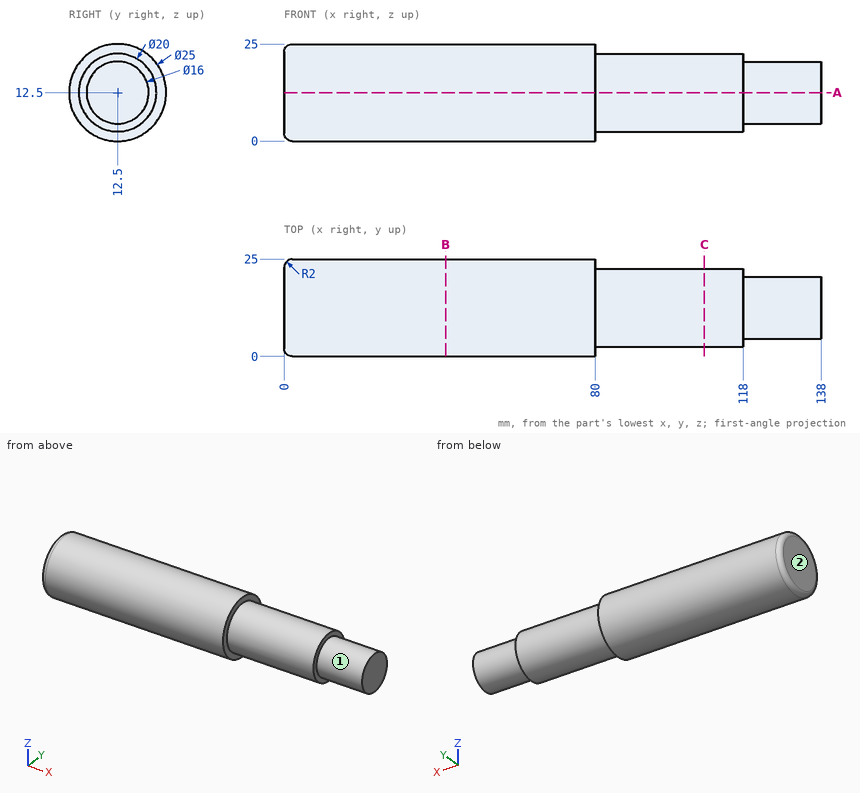
Job drawing, mm, ordinate dimensions from the low corner. One solid piece. A direction names the side the tool comes from. Round coordinates to 2 decimals unless told otherwise and drop trailing zeros. Order: outer loops, then holes, each group sorted by start corner. A loop starts at its lowest first (then second) coordinate and runs counter-clockwise, first axis right, second up. Notation, with made-up numbers: M 53.25,73.5 L 70.25,73.5 A11 ccw 70.25,94.5 Z; hole C 21,73.5 d2. An arc over 180 degrees is marked long. Write each question's results on one line, items separated by ' | '. Start each with the question number.
(1) Drop flat-ended pins along their axis: pin 1 (10 mm diameter, centred on y = 3.5, z = 7.5, fed in from -X); pin 2 (3 mm diameter, centred on x = 121.5, y = 8, fed in from +Z); pin 3 (1 mm diameter, centred on x = 114, z = 6.5, fed in from +Y); pin 4 (4 mm diameter, centred on x = 79.5, y = 5, fed in from -Z) (3 decimals). Give the stop position or say it passes through.
(2) Which spindle directions (+Z, -Z, +X, -X, +Y, -Y) get a long thin tool onto all of the face, cutting with end or side? Do the marked faces 1 and 2. Say none if no direction does.
(3) Saw through at A-A, the plane z = 12.5. Give the cut face in (x, y), then the cut area to 3 significant figures.
(4) Probe probe 1 along X at (y, z) = (16.5, 21.25); probe 2 along Y at (x, z) = (44.5, 5.75); probe 3 along X at (y, z) = (3, 16.5). List the from-to ranges inside material, lowest first. Write a range as from..to.
(5) Saw through at C-C, the plane x = 108. Give the cut face in (y, z).
(6) Saw through at B-B, the plane x = 41.5. Give the cut face in (y, z).
Established:
1) pin 1: stops at x = 0 | pin 2: stops at z = 19.92 | pin 3: stops at y = 20.85 | pin 4: stops at z = 1.275
2) face 1: +X | face 2: +Z, -Z, -X, +Y, -Y
3) outline: M 0,2 A2 ccw 2,0 L 80,0 L 80,2.5 L 118,2.5 L 118,4.5 L 138,4.5 L 138,20.5 L 118,20.5 L 118,22.5 L 80,22.5 L 80,25 L 2,25 A2 ccw 0,23 Z | area: 3,080 mm^2
4) probe 1: x = 0..118 | probe 2: y = 1.98..23.02 | probe 3: x = 0..80
5) outline: C 12.5,12.5 d20
6) outline: C 12.5,12.5 d25
